Geometry check sheet. Reference: the model listing, model coordinates, mm. Round coordinates to 2 decimals unless told otherwise and drop trailing zeros. Order: outer loops, then holes, each group sorted by start corner. A loop starts at its lowest first (then second) coordinate and runs counter-clockwise, first axis right, second up. Notation, with made-up numbers: (11, 4) - (66, 4) arc R33 ccw to (66, 37) - close; hole circle Ø1 at (-23, 5.25). An arc over 180 degrees is marked (long way). Return JSON: item names as keys, results as strings. Group by question number.
Q1. Sectioned sample at A-A, the plane y = 112.5. Record the cut outline in (x, z), then the cut area to 3 significant figures.
Q2. Material ranges on line 1 along Z through (x, y) = (3.65, -485); line 2 along Y through (x, z) = (1.7, 655); line 3 along Z through (x, y) = (1.55, -200), recorded low to high.
Q3. Gauge pin test, flat ends, axial feed: pin 1 Ø1.5 at (x, z) = (2, -652.5) entering from +Y; pin 2 Ø2.5 at (x, y) = (2, 133.5) entering from -Z. Record the tip position at first contact, or that the pin passes through.
```python
from build123d import *

# Parameters (mm, degrees)
SKETCH_1_W          = 1340
SKETCH_1_H          = 1000
EXTRUDE_1_DEPTH     = 5
CHAMFER_1_SIZE      = 1
SKETCH_2_R          = 3
CUT_EXTRUDE_1_DEPTH = 837.017344318
SKETCH_3_W          = 30
SKETCH_3_H          = 500
CUT_EXTRUDE_2_DEPTH = 10
CHAMFER_2_SIZE      = 1
FILLET_1_R          = 5
FILLET_2_R          = 5


with BuildPart() as part:
    # 草图1 → 凸台-拉伸1 (new body)
    with BuildSketch(Plane(origin=(0, 0, 0), x_dir=(0, 0, -1), z_dir=(1, 0, 0))):
        Rectangle(SKETCH_1_W, SKETCH_1_H)
    extrude(amount=EXTRUDE_1_DEPTH)

    # 倒角1
    chamfer_1_edges = [part.edges().sort_by_distance(p)[0] for p in [
        (2.5, 500, 670),
        (2.5, 500, -670),
        (2.5, -500, -670),
        (2.5, -500, 670),
    ]]
    chamfer(chamfer_1_edges, length=CHAMFER_1_SIZE)

    # 草图2 → 切除-拉伸1 (cut, through all)
    with BuildSketch(Plane.ZY):
        with Locations((-655, 485)):
            Circle(SKETCH_2_R)
        with Locations(Location((-655, -485, 0), (0, 0, 180))):
            Circle(SKETCH_2_R)
        with Locations((570, 485)):
            Circle(SKETCH_2_R)
        with Locations((655, 400)):
            Circle(SKETCH_2_R)
        with Locations((655, -400)):
            Circle(SKETCH_2_R)
        with Locations((570, -485)):
            Circle(SKETCH_2_R)
        with Locations((655, 0)):
            Circle(SKETCH_2_R)
        with Locations((-659, 200)):
            Circle(SKETCH_2_R)
        with Locations((-659, -200)):
            Circle(SKETCH_2_R)
    extrude(amount=-CUT_EXTRUDE_1_DEPTH, mode=Mode.SUBTRACT)

    # 草图3 → 切除-拉伸2 (cut)
    with BuildSketch(Plane(origin=(5, 0, 0), x_dir=(0, 0, -1), z_dir=(1, 0, 0))):
        with Locations((655, 250)):
            Rectangle(SKETCH_3_W, SKETCH_3_H)
    extrude(amount=-CUT_EXTRUDE_2_DEPTH, mode=Mode.SUBTRACT)

    # 倒角2
    chamfer_2_edges = [part.edges().sort_by_distance(p)[0] for p in [
        (2.5, 500, -640),
    ]]
    chamfer(chamfer_2_edges, length=CHAMFER_2_SIZE)

    # 圆角1
    fillet_1_edges = [part.edges().sort_by_distance(p)[0] for p in [
        (2.5, 0, -640),
    ]]
    fillet(fillet_1_edges, radius=FILLET_1_R)

    # 圆角2
    fillet_2_edges = [part.edges().sort_by_distance(p)[0] for p in [
        (2.5, 0, -670),
    ]]
    fillet(fillet_2_edges, radius=FILLET_2_R)


solid = part.part
```
Reply:
{
 "1": {"outline": "(0, -640) - (5, -640) - (5, 670) - (0, 670) - close", "area": "6,550 mm^2"},
 "2": {"line 1": "-670 to -658, -652 to 567, 573 to 670", "line 2": "-500 to -403, -397 to -3, 3 to 397, 403 to 500", "line 3": "-670 to -662, -656 to 670"},
 "3": {"pin 1": "y = 0", "pin 2": "z = -640"}
}
